from build123d import *

# Parameters (mm, degrees)
SKETCH1_R           = 10.5
SKETCH1_R_2         = 6
BOSS_EXTRUDE1_DEPTH = 30
FILLET1_R           = 1


with BuildPart() as part:
    # Sketch1 → Boss-Extrude1 (new body)
    with BuildSketch(Plane(origin=(0, 0, 0), x_dir=(1, 0, 0), z_dir=(0, 1, 0))):
        with Locations(Location((0, 0, 0), (0, 0, 270))):
            Circle(SKETCH1_R)
        with Locations(Location((0, 0, 0), (0, 0, 270))):
            Circle(SKETCH1_R_2, mode=Mode.SUBTRACT)
    extrude(amount=BOSS_EXTRUDE1_DEPTH)

    # Fillet1
    fillet1_edges = [part.edges().sort_by_distance(p)[0] for p in [
        (0, 0, -10.5),
        (0, 30, -10.5),
        (0, 0, -6),
        (0, 30, -6),
    ]]
    fillet(fillet1_edges, radius=FILLET1_R)


solid = part.part
Geometry check sheet. Reference: the model listing, model coordinates, mm. Give positions to 0.01 mm unless a question says otherwise; leave off trailing zeros. Order: outer loops, then holes, each group sorted by start corner. A loop starts at its lowest first (then second) coordinate and runs counter-clockwise, first axis right, second up.
1) Cross-section at B-B (x = 0). Record the boundary of the cut face in (y, z).
Results are:
outline: (0, -9.5) arc R1 ccw to (1, -10.5) - (29, -10.5) arc R1 ccw to (30, -9.5) - (30, -7) arc R1 ccw to (29, -6) - (1, -6) arc R1 ccw to (0, -7) - close; (0, 7) arc R1 ccw to (1, 6) - (29, 6) arc R1 ccw to (30, 7) - (30, 9.5) arc R1 ccw to (29, 10.5) - (1, 10.5) arc R1 ccw to (0, 9.5) - close
2) Material ranges on probe 1 along X at (y, z) = (23, 0); probe 2 along Z at (x, y) = (-4.75, 28.5); probe 3 along Z at (x, y) = (-0.25, 25.75), recorded low to high.
Results are:
probe 1: x = -10.5 to -6, 6 to 10.5
probe 2: z = -9.36 to -3.67, 3.67 to 9.36
probe 3: z = -10.5 to -5.99, 5.99 to 10.5
3) Cross-section at C-C (y = 15). Record the boundary of the cut face in (x, z).
Results are:
outline: circle Ø21 at (0, 0); hole circle Ø12 at (0, 0)
4) Gauge pin test, flat ends, axial feed: pin 1 (1 mm diameter, centred on x = 1, y = 15.5, fed in from +Z); pin 2 (1 mm diameter, centred on x = 5, y = 8, fed in from -Z); pin 3 (8 mm diameter, centred on y = 10, z = -7, fed in from +X); pin 4 (7 mm diameter, centred on x = 0, z = 0, fed in from +Y). Record the tip position at first contact, or that the pin passes through.
Results are:
pin 1: stops at z = 10.49
pin 2: stops at z = -9.49
pin 3: stops at x = 10.06
pin 4: passes through
5) Cross-section at A-A (z = 0). Record the boundary of the cut face in (x, y), then the cut area to 3 significant figures.
Results are:
outline: (-10.5, 1) arc R1 ccw to (-9.5, 0) - (-7, 0) arc R1 ccw to (-6, 1) - (-6, 29) arc R1 ccw to (-7, 30) - (-9.5, 30) arc R1 ccw to (-10.5, 29) - close; (6, 1) arc R1 ccw to (7, 0) - (9.5, 0) arc R1 ccw to (10.5, 1) - (10.5, 29) arc R1 ccw to (9.5, 30) - (7, 30) arc R1 ccw to (6, 29) - close
area: 268 mm2
6) Draft check along Z on faces 1 (the cylindrical face through (1.802, 14.804, 5.723)), 2 (the flat face through (-6, 30, -4)), 3 (the cylindrical face through (3.2, 14.8, 10)). Enter one of: released by +Z, released by -Z, zero draft, split by the parting line, or undercut.
Results are:
face 1: undercut
face 2: zero draft
face 3: split by the parting line
